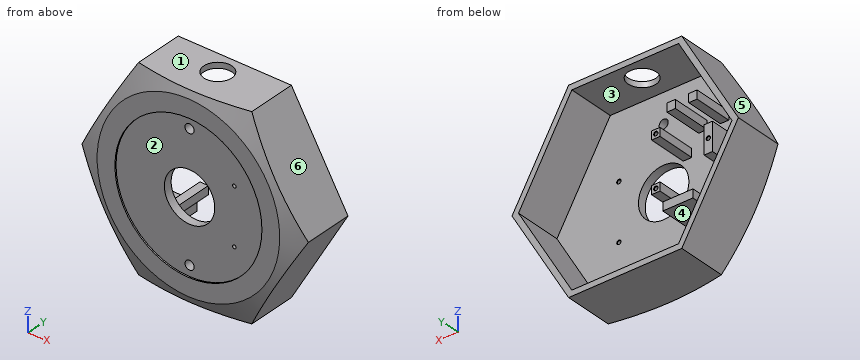
```python
from build123d import *

# Parameters (mm, degrees)
BOSS_EXTRUDE1_DEPTH         = 41
CUT_EXTRUDE1_DEPTH          = 34
SKETCH4_R                   = 52.5
CUT_EXTRUDE2_DEPTH          = 1
SKETCH5_W                   = 21.5
SKETCH5_H                   = 6
SKETCH5_W_2                 = 6
SKETCH5_H_2                 = 20
BOSS_EXTRUDE2_DEPTH         = 28
SKETCH6_R                   = 18
CUT_EXTRUDE3_DEPTH          = 28
SKETCH7_R                   = 3.25
CUT_EXTRUDE4_DEPTH          = 28
M3_TAPPED_HOLE1_D           = 2.5
M3_TAPPED_HOLE1_CSINK_D     = 3.05
M3_TAPPED_HOLE1_CSINK_ANGLE = 90
M3_TAPPED_HOLE2_D           = 2.5
M3_TAPPED_HOLE2_DEPTH       = 8
M3_TAPPED_HOLE2_CSINK_D     = 3.05
M3_TAPPED_HOLE2_CSINK_ANGLE = 90
M3_TAPPED_HOLE2_TIP         = 0.751075774
SKETCH8_R                   = 10
CUT_EXTRUDE5_DEPTH          = 28


with BuildPart() as part:
    # Sketch1 → Boss-Extrude1 (new body)
    with BuildSketch(Plane(origin=(0, 0, 0), x_dir=(1, 0, 0), z_dir=(0, 1, 0))):
        Polygon((-40.414518843, 70), (-80.829037687, 0), (-40.414518843, -70), (40.414518843, -70), (80.829037687, 0), (40.414518843, 70), align=None)
    extrude(amount=BOSS_EXTRUDE1_DEPTH)

    # Sketch2 → Cut-Extrude1 (cut)
    with BuildSketch(Plane(origin=(0, 41, 0), x_dir=(1, 0, 0), z_dir=(0, 1, 0))):
        Polygon((38.105117767, -66), (76.210235533, 0), (38.105117767, 66), (-38.105117767, 66), (-76.210235533, 0), (-38.105117767, -66), align=None)
    extrude(amount=-CUT_EXTRUDE1_DEPTH, mode=Mode.SUBTRACT)

    # Sketch3 → Cut-Revolve1 (revolve, cut)
    with BuildSketch(Plane.XY, mode=Mode.PRIVATE) as cut_revolve1_sk:
        Polygon((-80.829037687, 6), (-65.198503298, 0), (-80.829037687, 0), align=None)
    revolve(cut_revolve1_sk.sketch.rotate(Axis((0, 62.900603769, 0), (0, -1, 0)), 270), axis=Axis((0, 62.900603769, 0), (0, -1, 0)), mode=Mode.SUBTRACT)

    # Sketch4 → Cut-Extrude2 (cut)
    with BuildSketch(Plane.XZ):
        with Locations(Location((0, 0, 0), (0, 0, 270))):
            Circle(SKETCH4_R)
    extrude(amount=-CUT_EXTRUDE2_DEPTH, mode=Mode.SUBTRACT)

    # Sketch5 → Boss-Extrude2 (add)
    with BuildSketch(Plane(origin=(0, 7, 0), x_dir=(1, 0, 0), z_dir=(0, 1, 0))):
        with Locations((-32.75, 32)):
            Rectangle(SKETCH5_W, SKETCH5_H)
        with Locations((-54.5, 0)):
            Rectangle(SKETCH5_W_2, SKETCH5_H_2)
        with Locations((-43.5, -32)):
            Rectangle(SKETCH5_W_2, SKETCH5_H)
        with Locations((-28, -32)):
            Rectangle(SKETCH5_W_2, SKETCH5_H)
        with Locations((-17, 18)):
            Rectangle(SKETCH5_W_2, SKETCH5_H)
        with Locations((-17, -18)):
            Rectangle(SKETCH5_W_2, SKETCH5_H)
    extrude(amount=BOSS_EXTRUDE2_DEPTH)

    # Sketch6 → Cut-Extrude3 (cut)
    with BuildSketch(Plane(origin=(0, 7, 0), x_dir=(1, 0, 0), z_dir=(0, 1, 0))):
        with Locations(Location((0, 0, 0), (0, 0, 270))):
            Circle(SKETCH6_R)
    extrude(amount=-CUT_EXTRUDE3_DEPTH, mode=Mode.SUBTRACT)

    # Sketch7 → Cut-Extrude4 (cut)
    with BuildSketch(Plane(origin=(0, 7, 0), x_dir=(1, 0, 0), z_dir=(0, 1, 0))):
        with Locations(Location((0, 45, 0), (0, 0, 270))):
            Circle(SKETCH7_R)
        with Locations(Location((0, -45, 0), (0, 0, 90))):
            Circle(SKETCH7_R)
    extrude(amount=-CUT_EXTRUDE4_DEPTH, mode=Mode.SUBTRACT)

    # M3 Tapped Hole1 (through all)
    with Locations(Plane(origin=(0, 7, 0), x_dir=(1, 0, 0), z_dir=(0, 1, 0))):
        with Locations((32, 20), (32, -20)):
            CounterSinkHole(M3_TAPPED_HOLE1_D / 2, M3_TAPPED_HOLE1_CSINK_D / 2, counter_sink_angle=M3_TAPPED_HOLE1_CSINK_ANGLE)

    # M3 Tapped Hole2
    with Locations(Plane(origin=(0, 35, 0), x_dir=(1, 0, 0), z_dir=(0, 1, 0))):
        with Locations((-54.5, 0), (-17, 18), (-17, -18)):
            CounterSinkHole(M3_TAPPED_HOLE2_D / 2, M3_TAPPED_HOLE2_CSINK_D / 2, depth=M3_TAPPED_HOLE2_DEPTH, counter_sink_angle=M3_TAPPED_HOLE2_CSINK_ANGLE)
            with Locations((0, 0, -(M3_TAPPED_HOLE2_DEPTH + M3_TAPPED_HOLE2_TIP / 2))):  # 118° drill point
                Cone(0, M3_TAPPED_HOLE2_D / 2, M3_TAPPED_HOLE2_TIP, mode=Mode.SUBTRACT)

    # Sketch8 → Cut-Extrude5 (cut)
    with BuildSketch(Plane(origin=(0, 0, 66), x_dir=(-1, 0, 0), z_dir=(0, 0, -1))):
        with Locations((0, 26)):
            Circle(SKETCH8_R)
    extrude(amount=-CUT_EXTRUDE5_DEPTH, mode=Mode.SUBTRACT)


solid = part.part
```
Source: CAD feature listing. Evaluate the final solid. Frame: model axes, mm. Face numbers are marked on the shaded views. A direction names the side the tool comes from. Round coordinates to 2 decimals unless told otherwise and drop trailing zeros. Use a Markdown table: item, result. Add a question column.
1. Cut plane A-A, the plane y = 13. State how many separate pieces and enclosed holes the cut face has, and give its area (3 significant figures).
2. Set-up query: the marked faces 1, 2 and 3. Return all of +Z, -Z, +X, -X, +Y, -Y with unobstructed straight access to the full face (end or side cutting, diameter ignored); none if empty.
3. Ray query, line 1 along Z through (x, y) = (-27, 22.5); line 2 along Z through (x, y) = (-17, 30); line 3 along Z through (x, y) = (-13, 25.5). Return the intervals inside material, ascending. Write a range as [from, to].
4. Pull-direction query (X, two-part tool) for the marked faces 4, 5 and 6; classes: +X half, -X half, draft (parallel to the pull), parting line (faces both ways), or undercut.
5. Contact query for flat-ended pins moving along their axis: pin 1 (5 mm diameter, centred on x = -43.5, y = 16.5, fed in from +Z); pin 2 (2 mm diameter, centred on x = -58.5, y = 33, fed in from +Z); pin 3 (1 mm diameter, centred on y = 27, z = 41.5, fed in from -X); pin 4 (2 mm diameter, centred on x = 32, z = 20, fed in from +Y). Output: stop coordinate, or through.
Solution:
| question | item | result |
|---|---|---|
| 1 | separate pieces | 7 |
| 1 | enclosed holes | 1 |
| 1 | area | 2,280 mm2 |
| 2 | face 1 | +Z, +X, -X, +Y, -Y |
| 2 | face 2 | -Y |
| 2 | face 3 | +Y |
| 3 | line 1 | z = [-70, -66], [-35, -29], [29, 35], [66, 70] |
| 3 | line 2 | z = [-70, -66], [-21, -19.25], [-16.75, -15], [15, 16.75], [19.25, 21], [66, 70] |
| 3 | line 3 | z = [-70, -66], [66, 70] |
| 4 | face 4 | undercut |
| 4 | face 5 | -X half |
| 4 | face 6 | +X half |
| 5 | pin 1 | stops at z = 68.99 |
| 5 | pin 2 | stops at z = 40.41 |
| 5 | pin 3 | stops at x = -57.16 |
| 5 | pin 4 | passes through |
